The listing builds one solid part. Answer for the finished solid, in the listing's coordinates (mm). Face numbers are marked on the shaded views. A direction names the side the tool comes from. Give positions to 0.01 mm unless a question says otherwise; leave off trailing zeros. Write each loop counter-clockwise with the first axis right and the second up, starting at its lowest first coordinate (ties: lowest second). Pieces come first, ordered by that corner, then holes.
```python
from build123d import *

# Parameters (mm, degrees)
SKETCH_1_W                    = 520
SKETCH_1_H                    = 200
EXTRUDE_1_DEPTH               = 150
HOLE_WIZARD_M12_1_D           = 10.2
HOLE_WIZARD_M12_1_DEPTH       = 15
HOLE_WIZARD_M12_1_CSINK_D     = 12.05
HOLE_WIZARD_M12_1_CSINK_ANGLE = 90
HOLE_WIZARD_M12_1_TIP         = 3.064389157
CHAMFER_1_SIZE                = 10


with BuildPart() as part:
    # 草图1 → 凸台-拉伸1 (new body)
    with BuildSketch(Plane(origin=(0, 0, 0), x_dir=(1, 0, 0), z_dir=(0, 1, 0))):
        with Locations((-260, 100)):
            Rectangle(SKETCH_1_W, SKETCH_1_H)
    extrude(amount=EXTRUDE_1_DEPTH)

    # M12 螺纹孔1
    with Locations(Plane(origin=(0, 150, 0), x_dir=(1, 0, 0), z_dir=(0, 1, 0))):
        with Locations((-260, 100), (-173.397459622, 50), (-346.602540378, 50)):
            CounterSinkHole(HOLE_WIZARD_M12_1_D / 2, HOLE_WIZARD_M12_1_CSINK_D / 2, depth=HOLE_WIZARD_M12_1_DEPTH, counter_sink_angle=HOLE_WIZARD_M12_1_CSINK_ANGLE)
            with Locations((0, 0, -(HOLE_WIZARD_M12_1_DEPTH + HOLE_WIZARD_M12_1_TIP / 2))):  # 118° drill point
                Cone(0, HOLE_WIZARD_M12_1_D / 2, HOLE_WIZARD_M12_1_TIP, mode=Mode.SUBTRACT)

    # 草图6 → 切除-旋转1 (revolve, cut)
    with BuildSketch(Plane.XY):
        Polygon((-260, 150), (-340, 150), (-340, 122), (-385, 122), (-385, 93), (-400, 93), (-400, 81), (-385, 81), (-385, 15), (-370, 15), (-370, 0), (-260, 0), align=None)
    revolve(axis=Axis((-260, 0, 0), (0, 1, 0)), mode=Mode.SUBTRACT)

    # 倒角1
    chamfer_1_edges = [part.edges().sort_by_distance(p)[0] for p in [
        (-260, 122, -80),
    ]]
    chamfer(chamfer_1_edges, length=CHAMFER_1_SIZE)


solid = part.part
```
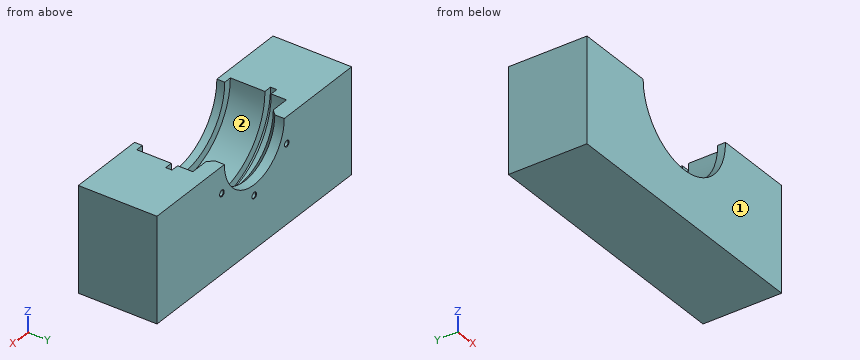
Item 1: Which of the six approach directions +Z, -Z, +X, -X, +Y, -Y give full straight-line access (tool end or side, diameter ignored) to the marked faces 1 and 2?
Conclusion:
face 1: +Z, -Z, +X, -X, -Y
face 2: +Z
Item 2: A cutting plane is placed at A-A, the plane y = 30.5. Give the vertices of the cut face in (x, z), plus the area to 3 significant figures.
Conclusion:
outline: (-520, -200) - (0, -200) - (0, 0) - (-135, 0) arc R125 cw to (-385, 0) - (-520, 0) - close
area: 79,500 mm2
Item 3: Each of these flat-tipped pins is pushed along its axis until it touches: P1, Ø10, axis at x = -299, y = 18, coming from the +Z side; P2, Ø11.5, axis at x = -173.4, z = -50, coming from the -Y side; P3, Ø6, axis at x = -182.5, y = 25.5, coming from the +Z side. Where does it stop, or does it pass through?
Conclusion:
P1: stops at z = -101.25
P2: stops at y = 122
P3: stops at z = -95.63
Item 4: Consider probe 1 along X at (y, z) = (140.5, -50); probe 2 along Y at (x, z) = (-204, -75.5); probe 3 along X at (y, z) = (41.5, -111.5). Determine where each line is inside the solid, lowest interval first.
Conclusion:
probe 1: x = -520 to -351.7, -341.5 to -322.45, -197.55 to -178.5, -168.3 to 0
probe 2: y = 122 to 150
probe 3: x = -520 to -316.5, -203.5 to 0
